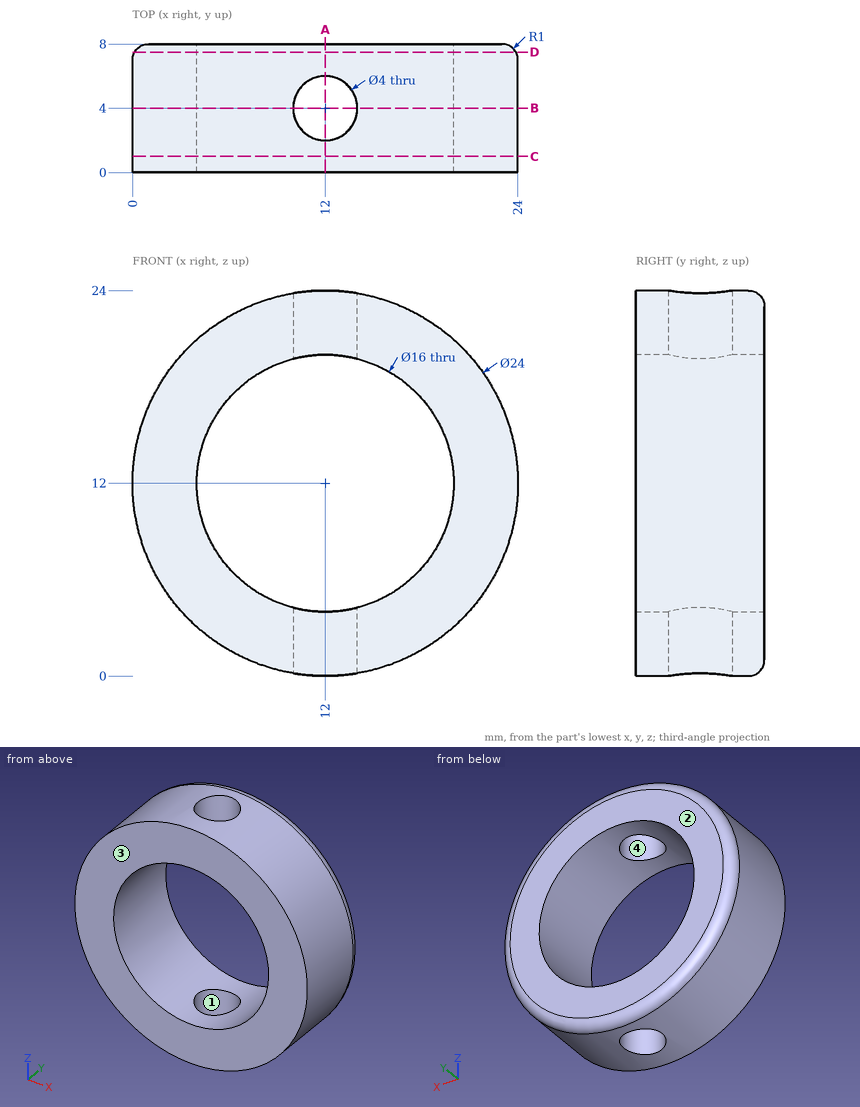
Print and shaded views of the part. All mm, measured from the part's lowest x, y and z. Round coordinates to 2 decimals unless told otherwise and drop trailing zeros. Write each loop counter-clockwise with the first axis right and the second up, starting at its lowest first coordinate (ties: lowest second). Pieces come first, ordered by that corner, then holes. Notation, with made-up numbers: (83, 3.25) - (132, 3.25) arc R18 cw to (132, 7.25) - close; hole circle Ø3 at (-37, 85). An arc over 180 degrees is marked (long way). Write each question's results on one line, items separated by ' | '. Start each with the question number.
Item 1: Saw through at C-C (y = 1). Write the cut outline in (x, z).
Item 2: Saw through at A-A (x = 12). State how many separate pieces and enclosed holes the cut face has, and give its area (3 significant figures).
Item 3: Drop flat-ended pins along their axis: P1, Ø4, axis at y = 5.5, z = 5, coming from the +X side; P2, Ø3, axis at x = 10, y = 4, coming from the +Z side; P3, Ø1, axis at x = 7, y = 6.5, coming from the -Z side. Give the stop position or say it passes through.
Item 4: Wall check: L1, parallel to X at y = 5.75, z = 7 (3 decimals); L2, parallel to Z at x = 15.5, y = 6.25; L3, parallel to X at y = 2, z = 11.25. Give the ranges that are in metal, low to high. Write a range as [from, to].
Item 5: Saw through at B-B (y = 4). Write the cut outline in (x, z).
Item 6: Saw through at D-D (y = 7.5). Write the cut outline in (x, z).
Item 7: Mould opens along Y. For the marked faces 1, 2, 3 and 4 say: pulls with the +Y half, pulls with the -Y half, needs draft (parallel to the pull), parting line crosses it, or undercut.
Results are:
1) outline: circle Ø24 at (12, 12); hole circle Ø16 at (12, 12)
2) separate pieces: 4 | enclosed holes: 0 | area: 31.6 mm²
3) P1: stops at x = 22.91 | P2: stops at z = 23.91 | P3: stops at z = 0.88
4) L1: x = [1.091, 5.755], [18.245, 22.909] | L2: z = [0.52, 4.81], [19.19, 23.48] | L3: x = [0.02, 4.04], [19.96, 23.98]
5) outline: (10, 0.17) - (10, 4.25) arc R8 cw to (10, 19.75) - (10, 23.83) arc R12 ccw to start; (14, 0.17) arc R12 ccw to (14, 23.83) - (14, 19.75) arc R8 cw to (14, 4.25) - close
6) outline: circle Ø23.73 at (12, 12); hole circle Ø16 at (12, 12)
7) face 1: undercut | face 2: pulls with the +Y half | face 3: pulls with the -Y half | face 4: undercut
